The listing builds one solid part. Answer for the finished solid, in the listing's coordinates (mm). A direction names the side the tool comes from. Round coordinates to 2 decimals unless told otherwise and drop trailing zeros. Write each loop counter-clockwise with the first axis right and the second up, starting at its lowest first coordinate (ties: lowest second). Pieces come first, ordered by that corner, then holes. Notation, with made-up numbers: (-32.5, -8.75) - (19.5, -8.75) arc R11 ccw to (19.5, 8.25) - close; hole circle Ø4 at (-3, -4). An arc over 180 degrees is marked (long way). Return JSON: item names as keys, results as strings. Group by question number.
(1) Section A-A, the plane z = 0 is taken. Write down the section's boundary in (x, y).
(2) Which of the six approach directions +Z, -Z, +X, -X, +Y, -Y give full straight-line access (tool end or side, diameter ignored) to faces 4 (the flat face through (-34.25, 7, 0)), 5 (the flat face through (24, 0.7, 4)), 6 (the flat face through (-23.25, 12.8, 0.1))?
(3) Each of these flat-tipped pins is pushed along its axis until it touches: pin 1 (9 mm diameter, centred on x = -12.75, z = 0, fed in from +Y); pin 2 (4 mm diameter, centred on y = 15.5, z = 0, fed in from -X); pin 3 (7 mm diameter, centred on y = 11.5, z = -1.5, fed in from +X); pin 4 (7.5 mm diameter, centred on x = 17.5, z = 2, fed in from +Y). Where does it stop, or does it pass through?
(4) Determine the mould class of faces 1 (the flat face through (-8, 3, -7.5)), 2 (the cylindrical face through (-9.453, -3.457, -0.145)), 3 (the flat face through (34.25, 0, 0)) for opening direction Z: +Z half, -Z half, draft (parallel to the pull), parting line (faces both ways), or undercut.
(5) Section C-C, the plane x = 24.25 is taken. Write down the section's boundary in (y, z), then the cut area to 3 significant figures.
(6) Find the intervals of material crossed by line 1 along X through (y, z) = (-4, -3); line 2 along X through (y, z) = (-0.25, -1); line 3 along Z through (x, y) = (-12.75, 4.5), in increasing order. Write a range as [from, to].
(7) Section D-D, the plane y = 15.5 is taken. Write down the section's boundary in (x, z), then the cut area to 3 significant figures.
(8) Section B-B, the plane y = -4 is taken. Write down the section's boundary in (x, z), then the cut area to 3 significant figures.
```python
from build123d import *

# Parameters (mm, degrees)
SKETCH_1_W                   = 68.5
SKETCH_1_H                   = 15
EXTRUDE_1_DEPTH              = 7.5
SKETCH_2_W                   = 11
SKETCH_2_H                   = 15
EXTRUDE_2_DEPTH              = 14
CHAMFER_1_SIZE               = 1
HOLE_WIZARD_M6_1_D           = 6.6
HOLE_WIZARD_M6_1_CBORE_D     = 11
HOLE_WIZARD_M6_1_CBORE_DEPTH = 6.8
HOLE_WIZARD_M6_1_2_D         = 5


with BuildPart() as part:
    # 草图1 → 凸台-拉伸1 (new, symmetric)
    with BuildSketch(Plane(origin=(0, 0, 0), x_dir=(1, 0, 0), z_dir=(0, 1, 0))):
        Rectangle(SKETCH_1_W, SKETCH_1_H)
    extrude(amount=EXTRUDE_1_DEPTH, both=True)

    # 草图2 → 凸台-拉伸2 (add)
    with BuildSketch(Plane(origin=(0, 7.5, 0), x_dir=(1, 0, 0), z_dir=(0, 1, 0))):
        with Locations((-28.75, 0)):
            Rectangle(SKETCH_2_W, SKETCH_2_H)
    extrude(amount=EXTRUDE_2_DEPTH)

    # 倒角1
    chamfer_1_edges = [part.edges().sort_by_distance(p)[0] for p in [
        (-28.75, 21.5, 7.5),
        (-28.75, 21.5, -7.5),
        (-34.25, -7.5, 0),
        (34.25, 0, 7.5),
        (34.25, 0, -7.5),
    ]]
    chamfer(chamfer_1_edges, length=CHAMFER_1_SIZE)

    # Hole Wizard M6 _1 (through all)
    with Locations(Plane(origin=(0, 7.5, 0), x_dir=(1, 0, 0), z_dir=(0, 1, 0))):
        with Locations((24.25, 0), (-12.75, 0)):
            CounterBoreHole(HOLE_WIZARD_M6_1_D / 2, HOLE_WIZARD_M6_1_CBORE_D / 2, HOLE_WIZARD_M6_1_CBORE_DEPTH)

    # Hole Wizard M6 _1 2 (through all)
    with Locations(Plane.ZY.offset(34.25)):
        with Locations((0, 15.5)):
            Hole(HOLE_WIZARD_M6_1_2_D / 2)


solid = part.part
```
Working result:
{
 "1": {"outline": "(-34.25, -6.5) - (-33.25, -7.5) - (-16.05, -7.5) - (-16.05, 0.7) - (-18.25, 0.7) - (-18.25, 7.5) - (-23.25, 7.5) - (-23.25, 13) - (-34.25, 13) - close; (-34.25, 18) - (-23.25, 18) - (-23.25, 21.5) - (-34.25, 21.5) - close; (-9.45, -7.5) - (20.95, -7.5) - (20.95, 0.7) - (18.75, 0.7) - (18.75, 7.5) - (-7.25, 7.5) - (-7.25, 0.7) - (-9.45, 0.7) - close; (27.55, -7.5) - (34.25, -7.5) - (34.25, 7.5) - (29.75, 7.5) - (29.75, 0.7) - (27.55, 0.7) - close"},
 "2": {"face 4": "+Z, -Z, -X, +Y, -Y", "face 5": "+Y", "face 6": "+Z, -Z, +X, +Y"},
 "3": {"pin 1": "stops at y = 0.7", "pin 2": "passes through", "pin 3": "stops at x = -23.25", "pin 4": "stops at y = 7.5"},
 "4": {"face 1": "-Z half", "face 2": "undercut", "face 3": "draft"},
 "5": {"outline": "(-7.5, -7.5) - (7.5, -7.5) - (7.5, -5.5) - (0.7, -5.5) - (0.7, -3.3) - (-7.5, -3.3) - close; (-7.5, 3.3) - (0.7, 3.3) - (0.7, 5.5) - (7.5, 5.5) - (7.5, 7.5) - (-7.5, 7.5) - close", "area": "96.1 mm^2"},
 "6": {"line 1": "x = [-34.25, -14.12], [-11.38, 22.88], [25.62, 34.25]", "line 2": "x = [-34.25, -15.89], [-9.61, 21.11], [27.39, 34.25]", "line 3": "z = [-7.5, -5.5], [5.5, 7.5]"},
 "7": {"outline": "(-34.25, -7.5) - (-23.25, -7.5) - (-23.25, -2.5) - (-34.25, -2.5) - close; (-34.25, 2.5) - (-23.25, 2.5) - (-23.25, 7.5) - (-34.25, 7.5) - close", "area": "110 mm^2"},
 "8": {"outline": "(-34.25, -7.5) - (33.25, -7.5) - (34.25, -6.5) - (34.25, 6.5) - (33.25, 7.5) - (-34.25, 7.5) - close; hole circle Ø6.6 at (-12.75, 0); hole circle Ø6.6 at (24.25, 0)", "area": "958 mm^2"}
}
